from build123d import *

# Parameters (mm, degrees)
EXTRUDE_1_DEPTH     = 50
SKETCH_2_R          = 2.25
CUT_EXTRUDE_1_DEPTH = 10


with BuildPart() as part:
    # 草图1 → 拉伸-薄壁1 (new body)
    with BuildSketch(Plane.XY):
        Polygon((0, 0), (0, 25), (95, 25), (95, 22), (3, 22), (3, 0), align=None)
    extrude(amount=EXTRUDE_1_DEPTH)

    # 草图2 → 切除-拉伸1 (cut)
    with BuildSketch(Plane(origin=(3, 0, 0), x_dir=(0, 0, -1), z_dir=(1, 0, 0))):
        with Locations((-40, 11)):
            Circle(SKETCH_2_R)
        with Locations(Location((-10, 11, 0), (0, 0, 180))):
            Circle(SKETCH_2_R)
    extrude(amount=-CUT_EXTRUDE_1_DEPTH, mode=Mode.SUBTRACT)


solid = part.part
Geometry check sheet. Reference: the model listing, model coordinates, mm. A direction names the side the tool comes from. Give positions to 0.01 mm unless a question says otherwise; leave off trailing zeros. Order: outer loops, then holes, each group sorted by start corner. A loop starts at its lowest first (then second) coordinate and runs counter-clockwise, first axis right, second up.
1) Cross-section at D-D (y = 6). Record the boundary of the cut face in (x, z).
Results are:
outline: (0, 0) - (3, 0) - (3, 50) - (0, 50) - close
2) Draft check along Y on faces 3 (the flat face through (47, 25, 25)), 4 (the cylindrical face through (1.52, 9.48, 8.34)), 5 (the flat face through (50, 22, 25)), 6 (the flat face through (37, 24, 0)). Enter one of: released by +Y, released by -Y, zero draft, split by the parting line, or undercut.
Results are:
face 3: released by +Y
face 4: undercut
face 5: released by -Y
face 6: zero draft
3) Cross-section at A-A (z = 10). Record the boundary of the cut face in (x, y).
Results are:
outline: (0, 0) - (3, 0) - (3, 8.75) - (0, 8.75) - close; (0, 13.25) - (3, 13.25) - (3, 22) - (95, 22) - (95, 25) - (0, 25) - close
4) Cross-section at C-C (z = 32). Record the boundary of the cut face in (x, y), then the cut area to 3 significant figures.
Results are:
outline: (0, 0) - (3, 0) - (3, 22) - (95, 22) - (95, 25) - (0, 25) - close
area: 351 mm2
5) Cross-section at B-B (y = 11). Record the boundary of the cut face in (x, z), then the cut area to 3 significant figures.
Results are:
outline: (0, 0) - (3, 0) - (3, 7.75) - (0, 7.75) - close; (0, 12.25) - (3, 12.25) - (3, 37.75) - (0, 37.75) - close; (0, 42.25) - (3, 42.25) - (3, 50) - (0, 50) - close
area: 123 mm2
6) Material ranges on probe 1 along Y at (x, z) = (1, 10); probe 2 along Y at (x, z) = (62, 11); probe 3 along X at (y, z) = (3, 23.5), recorded low to high.
Results are:
probe 1: y = 0 to 8.75, 13.25 to 25
probe 2: y = 22 to 25
probe 3: x = 0 to 3
7) Gauge pin test, flat ends, axial feed: pin 1 (11 mm diameter, centred on y = 15.5, z = 24, fed in from +X); pin 2 (5 mm diameter, centred on x = 12, y = 18, fed in from +Z). Record the tip position at first contact, or that the pin passes through.
Results are:
pin 1: stops at x = 3
pin 2: passes through
8) Tool access check on faces 1 (the flat face through (95, 24, 25)), 2 (the flat face through (3, 11, 25)). Record the directions out of +Z, -Z, +X, -X, +Y, -Y that give a thin tool (end or side, any length) a straight path to the whole face; none if there is none.
Results are:
face 1: +Z, -Z, +X, +Y, -Y
face 2: +Z, -Z, +X, -Y
